```python
from build123d import *

# Parameters (mm, degrees)
BASE_PLATE_DEPTH            = 960
UPRIGHT_SKETCH_W            = 600
UPRIGHT_SKETCH_H            = 160
UPRIGHT_DEPTH               = 500
UPRIGHT_TOP_ROUND_R200_R    = 200
BORE_COUNTERBORE_SKETCH_R   = 100
BORE_COUNTERBORE_200_DEPTH  = 80
THROUGH_BORE_SKETCH_R       = 50
THROUGH_BORE_100_DEPTH      = 1223.456543195
MOUNTING_HOLES_SKETCH_R     = 42.5
MOUNTING_HOLES_2X_85_DEPTH  = 1238.578280352
BASE_POCKET_30_DEEP_DEPTH   = 30
POCKET_HOLE_SKETCH_R        = 42.5
POCKET_HOLE_85_DEPTH        = 30
FORK_SUPPORT_BLOCK_SKETCH_W = 130
FORK_SUPPORT_BLOCK_SKETCH_H = 300
FORK_SUPPORT_BLOCK_DEPTH    = 400
FORK_CRADLE_SKETCH_R        = 150
FORK_CRADLE_300_DEPTH       = 400
GUSSET_RIB_DEPTH            = 100


with BuildPart() as part:
    # Base Plate Profile Sketch → Base Plate (new body)
    with BuildSketch(Plane.XY):
        Polygon((0, 0), (100, 0), (100, 40), (220, 40), (220, 60), (380, 60), (380, 40), (500, 40), (500, 0), (600, 0), (600, 100), (0, 100), align=None)
    extrude(amount=-BASE_PLATE_DEPTH)

    # Upright Sketch → Upright (add)
    with BuildSketch(Plane(origin=(0, 100, 0), x_dir=(1, 0, 0), z_dir=(0, 1, 0))):
        with Locations((300, 880)):
            Rectangle(UPRIGHT_SKETCH_W, UPRIGHT_SKETCH_H)
    extrude(amount=UPRIGHT_DEPTH)

    # Upright Top Round R200
    upright_top_round_r200_edges = [part.edges().sort_by_distance(p)[0] for p in [
        (0, 600, -880),
    ]]
    fillet(upright_top_round_r200_edges, radius=UPRIGHT_TOP_ROUND_R200_R)

    # Bore Counterbore Sketch → Bore Counterbore Ø200 (cut)
    with BuildSketch(Plane.XY.offset(-800)):
        with Locations((200, 400)):
            Circle(BORE_COUNTERBORE_SKETCH_R)
    extrude(amount=-BORE_COUNTERBORE_200_DEPTH, mode=Mode.SUBTRACT)

    # Through Bore Sketch → Through Bore Ø100 (cut, through all)
    with BuildSketch(Plane.XY.offset(-880)):
        with Locations((200, 400)):
            Circle(THROUGH_BORE_SKETCH_R)
    extrude(amount=-THROUGH_BORE_100_DEPTH, mode=Mode.SUBTRACT)

    # Mounting Holes Sketch → Mounting Holes 2xØ85 (cut, through all)
    with BuildSketch(Plane(origin=(0, 100, 0), x_dir=(1, 0, 0), z_dir=(0, 1, 0))):
        with Locations(Location((120, 700, 0), (0, 0, 270))):
            Circle(MOUNTING_HOLES_SKETCH_R)
        with Locations(Location((120, 100, 0), (0, 0, 270))):
            Circle(MOUNTING_HOLES_SKETCH_R)
    extrude(amount=-MOUNTING_HOLES_2X_85_DEPTH, mode=Mode.SUBTRACT)

    # Base Pocket Sketch → Base Pocket 30 Deep (cut)
    with BuildSketch(Plane(origin=(0, 100, 0), x_dir=(1, 0, 0), z_dir=(0, 1, 0))):
        with BuildLine():
            Line((200, 300), (200, 0))
            Line((200, 0), (400, 0))
            Line((400, 0), (400, 300))
            ThreePointArc((400, 300), (300, 400), (200, 300))
        make_face()
    extrude(amount=-BASE_POCKET_30_DEEP_DEPTH, mode=Mode.SUBTRACT)

    # Pocket Hole Sketch → Pocket Hole Ø85 (cut)
    with BuildSketch(Plane(origin=(0, 70, 0), x_dir=(1, 0, 0), z_dir=(0, 1, 0))):
        with Locations(Location((300, 300, 0), (0, 0, 270))):
            Circle(POCKET_HOLE_SKETCH_R)
    extrude(amount=-POCKET_HOLE_85_DEPTH, mode=Mode.SUBTRACT)

    # Fork Support Block Sketch → Fork Support Block (add)
    with BuildSketch(Plane.XY.offset(-800)):
        with Locations((535, 250)):
            Rectangle(FORK_SUPPORT_BLOCK_SKETCH_W, FORK_SUPPORT_BLOCK_SKETCH_H)
    extrude(amount=FORK_SUPPORT_BLOCK_DEPTH)

    # Fork Cradle Sketch → Fork Cradle Ø300 (cut)
    with BuildSketch(Plane(origin=(600, 0, 0), x_dir=(0, 0, -1), z_dir=(1, 0, 0))):
        with Locations((600, 400)):
            Circle(FORK_CRADLE_SKETCH_R)
    extrude(amount=-FORK_CRADLE_300_DEPTH, mode=Mode.SUBTRACT)

    # Gusset Rib Sketch → Gusset Rib (add)
    with BuildSketch(Plane(origin=(600, 0, 0), x_dir=(0, 0, -1), z_dir=(1, 0, 0))):
        Polygon((400, 400), (400, 100), (0, 100), align=None)
    extrude(amount=-GUSSET_RIB_DEPTH)


solid = part.part
```
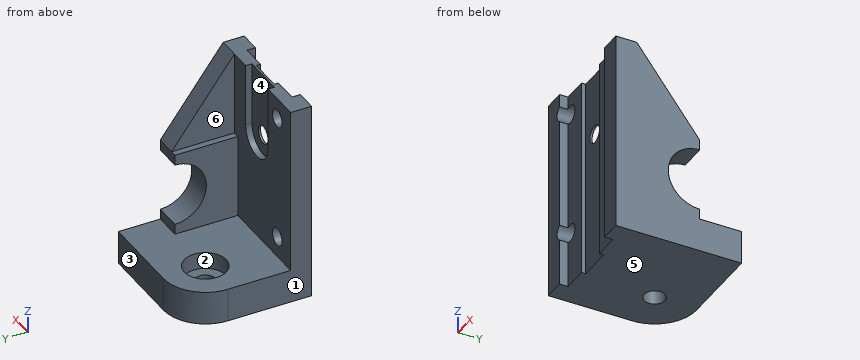
The listing builds one solid part. Answer for the finished solid, in the listing's coordinates (mm). Face numbers are marked on the shaded views. A direction names the side the tool comes from. Give positions to 0.01 mm unless a question says otherwise; leave off trailing zeros. Order: outer loops, then holes, each group sorted by start corner. A loop starts at its lowest first (then second) coordinate and runs counter-clockwise, first axis right, second up.
1) Find section D-D on z = -600. Write down the section's boundary in (x, y).
Reported:
outline: (0, 0) - (100, 0) - (100, 40) - (220, 40) - (220, 60) - (380, 60) - (380, 40) - (500, 40) - (500, 0) - (600, 0) - (600, 250) - (470, 250) - (470, 100) - (0, 100) - close
2) Find section C-C on x = 120. Write down the section's boundary in (y, z), then the cut area to 3 significant figures.
Reported:
outline: (40, -960) - (583.3, -960) - (583.3, -800) - (460, -800) - (460, -880) - (340, -880) - (340, -800) - (100, -800) - (100, -742.5) - (40, -742.5) - close; (40, -657.5) - (100, -657.5) - (100, -142.5) - (40, -142.5) - close; (40, -57.5) - (100, -57.5) - (100, 0) - (40, 0) - close
area: 115,000 mm2
3) Determine the mould class of the marked faces 1, 2 and 3 for opening direction Y: pulls with the +Y half, pulls with the -Y half, needs draft (parallel to the pull), parting line crosses it, or undercut.
Reported:
face 1: needs draft
face 2: undercut
face 3: pulls with the +Y half
4) Find section A-A on z = -100. Write down the section's boundary in (x, y).
Reported:
outline: (0, 0) - (77.5, 0) - (77.5, 100) - (0, 100) - close; (162.5, 40) - (220, 40) - (220, 60) - (380, 60) - (380, 40) - (500, 40) - (500, 0) - (600, 0) - (600, 175) - (500, 175) - (500, 100) - (400, 100) - (400, 70) - (200, 70) - (200, 100) - (162.5, 100) - close
5) Consider line 1 along Z through (x, y) = (120, 56); line 2 along Z through (x, y) = (90, 460); line 3 along Y through (x, z) = (43, -111). Determine where each line is inside the solid, lowest interval first.
Reported:
line 1: z = -960 to -742.5, -657.5 to -142.5, -57.5 to 0
line 2: z = -960 to -800
line 3: y = 0 to 100
6) Given P1, Ø6, axis at x = 393, y = 347.5, coming from the +Z side; P2, Ø5, axis at x = 380, z = -589.5, coming from the -Y side; P3, Ø12, axis at x = 308.5, z = -672, coming from the +Y side, each flat-ended and moving along its own axis, determine where each tip first touches the part or whether it passes through.
Reported:
P1: stops at z = -800
P2: stops at y = 40
P3: stops at y = 100
7) Find section B-B on z = -899. Write down the section's boundary in (x, y).
Reported:
outline: (0, 0) - (100, 0) - (100, 40) - (220, 40) - (220, 60) - (380, 60) - (380, 40) - (500, 40) - (500, 0) - (600, 0) - (600, 600) - (200, 600) arc R200 ccw to (0, 400) - close; hole circle Ø100 at (200, 400)
8) For the marked faces 4, 5 and 6, determine the directions among +Z, -Z, +X, -X, +Y, -Y from which every point of the face is accessible in a straight line to the end or side of a thin tool.
Reported:
face 4: +Z, +Y
face 5: -Z, +X, -X, +Y, -Y
face 6: +Z, -X, +Y
